Could you check a few things on this drawing? It's one solid part, dimensions in mm from its lowest x, y, z. Give positions to 0.01 mm unless a question says otherwise; leave off trailing zeros. Order: outer loops, then holes, each group sorted by start corner. A loop starts at its lowest first (then second) coordinate and runs counter-clockwise, first axis right, second up. Notation, with made-up numbers: (46.25, -17.5) -> (64.25, -17.5) arc R8 cw to (64.25, -3.5) -> close; hole circle Ø6 at (-32, 48.25). An arc over 180 degrees is marked (long way). Write each question's results on one line, items separated by ' | '.
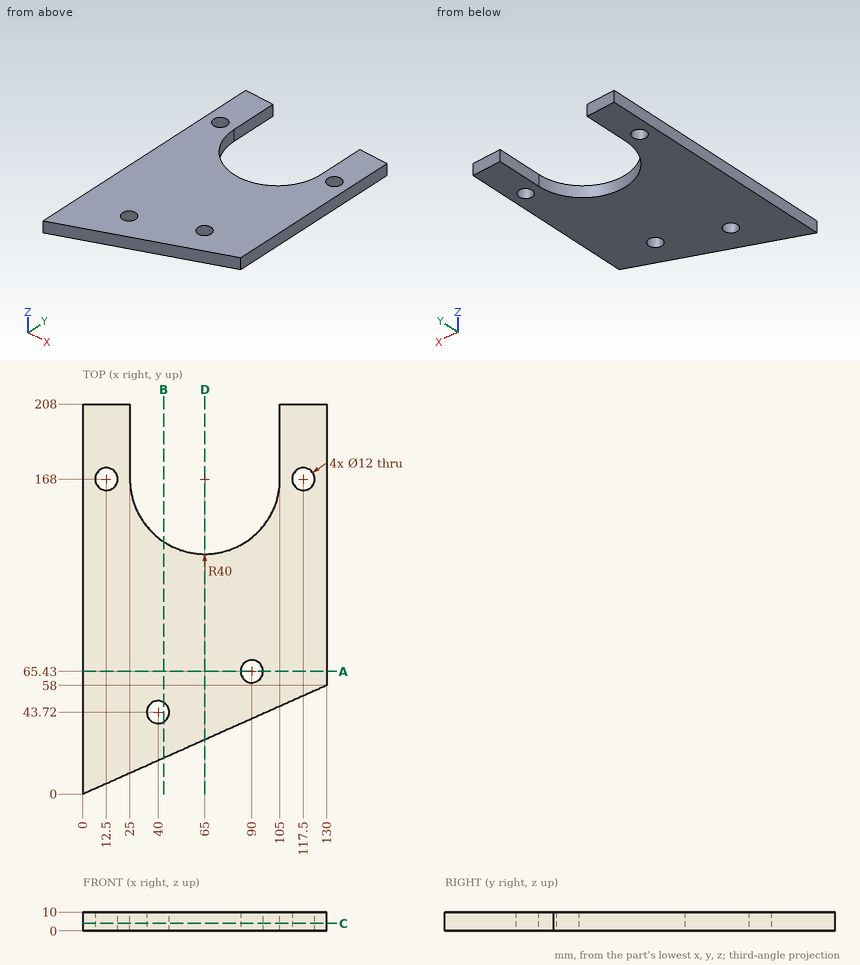
Q1. Suppose I cut it at C-C on z = 4. Please give me the cut outline in (x, y), and give its area (3 significant figures).
Here are the results:
outline: (0, 0) -> (130, 58) -> (130, 208) -> (105, 208) -> (105, 168) arc R40 cw to (25, 168) -> (25, 208) -> (0, 208) -> close; hole circle Ø12 at (12.5, 168); hole circle Ø12 at (40, 43.72); hole circle Ø12 at (90, 65.43); hole circle Ø12 at (117.5, 168) | area: 17,100 mm²
Q2. I need wall thicknesses on line 1 along X through (y, z) = (173.5, 7.5); line 2 along X through (y, z) = (169, 1); line 3 along Y through (x, z) = (117.5, 6.5). Which ranges of each line are inside material? Lowest first, please.
Here are the results:
line 1: x = 0 to 10.1, 14.9 to 25, 105 to 115.1, 119.9 to 130 | line 2: x = 0 to 6.58, 18.42 to 25, 105 to 111.58, 123.42 to 130 | line 3: y = 52.42 to 162, 174 to 208
Q3. Suppose I cut it at A-A on y = 65.43. Please give me the cut outline in (x, z), and give its area (3 significant figures).
Here are the results:
outline: (0, 0) -> (84, 0) -> (84, 10) -> (0, 10) -> close; (96, 0) -> (130, 0) -> (130, 10) -> (96, 10) -> close | area: 1,180 mm²
Q4. Suppose I cut it at D-D on x = 65. Please give me the cut outline in (y, z), and give its area (3 significant figures).
Here are the results:
outline: (29, 0) -> (128, 0) -> (128, 10) -> (29, 10) -> close | area: 990 mm²
Q5. Suppose I cut it at B-B on x = 43. Please give me the cut outline in (y, z), and give its area (3 significant figures).
Here are the results:
outline: (19.18, 0) -> (38.52, 0) -> (38.52, 10) -> (19.18, 10) -> close; (48.92, 0) -> (134.59, 0) -> (134.59, 10) -> (48.92, 10) -> close | area: 1,050 mm²
